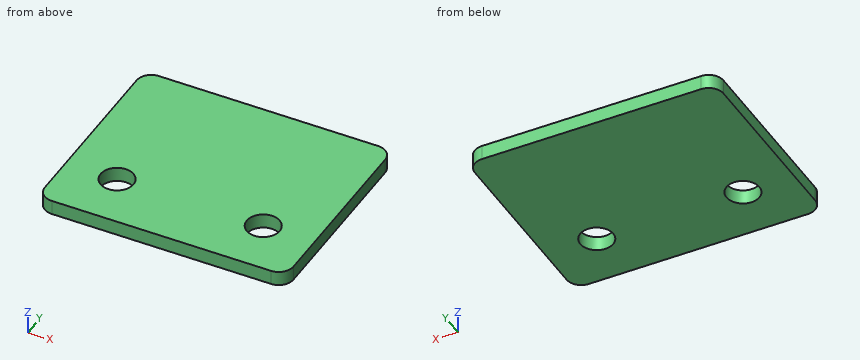
from build123d import *

# Parameters (mm, degrees)
SKETCH1_W           = 34
SKETCH1_H           = 28
SKETCH1_R           = 2.25
BOSS_EXTRUDE1_DEPTH = 2
FILLET1_R           = 2


with BuildPart() as part:
    # Sketch1 → Boss-Extrude1 (new body)
    with BuildSketch(Plane.XY):
        with Locations((0, 14)):
            Rectangle(SKETCH1_W, SKETCH1_H)
        with Locations((-10, 7.5)):
            Circle(SKETCH1_R, mode=Mode.SUBTRACT)
        with Locations(Location((10, 7.5, 0), (0, 0, 180))):
            Circle(SKETCH1_R, mode=Mode.SUBTRACT)
    extrude(amount=BOSS_EXTRUDE1_DEPTH)

    # Fillet1
    fillet1_edges = [part.edges().sort_by_distance(p)[0] for p in [
        (17, 0, 1),
        (-17, 0, 1),
        (-17, 28, 1),
        (17, 28, 1),
    ]]
    fillet(fillet1_edges, radius=FILLET1_R)


solid = part.part
The model under review builds one solid part; all positions refer to its coordinate system, in mm. Coordinates: 2 decimals unless noted, no trailing zeros. Loops run counter-clockwise (first coordinate to the right, second up) from the corner with the lowest first, then second, coordinate; pieces in that order, holes last.
(1) Consider section B-B, the plane x = -10. Give the boundary of the cut face in (y, z).
Determined:
outline: (0, 0) - (5.25, 0) - (5.25, 2) - (0, 2) - close; (9.75, 0) - (28, 0) - (28, 2) - (9.75, 2) - close
(2) Consider section A-A, the plane y = 7.5. Give the boundary of the cut face in (x, z), plus the area to 3 significant figures.
Determined:
outline: (-17, 0) - (-12.25, 0) - (-12.25, 2) - (-17, 2) - close; (-7.75, 0) - (7.75, 0) - (7.75, 2) - (-7.75, 2) - close; (12.25, 0) - (17, 0) - (17, 2) - (12.25, 2) - close
area: 50.0 mm2
(3) Consider section C-C, the plane z = 1.7. Give the boundary of the cut face in (x, y).
Determined:
outline: (-17, 2) arc R2 ccw to (-15, 0) - (15, 0) arc R2 ccw to (17, 2) - (17, 26) arc R2 ccw to (15, 28) - (-15, 28) arc R2 ccw to (-17, 26) - close; hole circle Ø4.5 at (-10, 7.5); hole circle Ø4.5 at (10, 7.5)
(4) Wall thickness on L1, parallel to Y at x = -10, z = 1.35; L2, parallel to X at y = 6, z = 1.25; L3, parallel to Y at x = -11, z = 1.4: over which ranges is each line inside the solid? List them lowest first.
Determined:
L1: y = 0 to 5.25, 9.75 to 28
L2: x = -17 to -11.68, -8.32 to 8.32, 11.68 to 17
L3: y = 0 to 5.48, 9.52 to 28
